Part model, mm, in its own coordinate system. Face numbers are marked on the shaded views. A direction names the side the tool comes from. Give positions to 0.01 mm unless a question says otherwise; leave off trailing zeros. Order: outer loops, then holes, each group sorted by start corner. A loop starts at its lowest first (then second) coordinate and runs counter-clockwise, first axis right, second up.
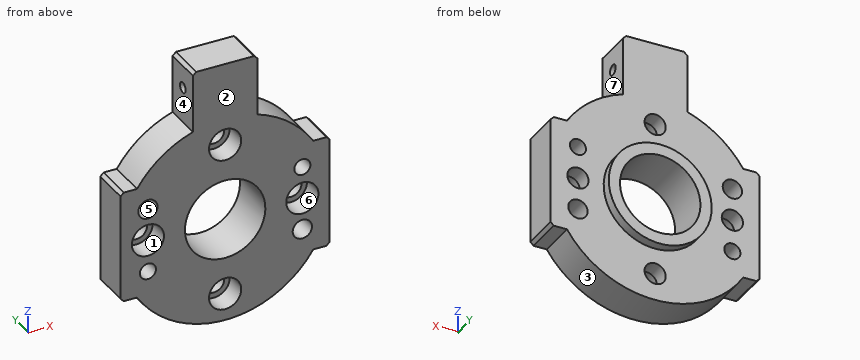
from build123d import *

# Parameters (mm, degrees)
EXTRUDE_1_DEPTH              = 15
SKETCH_2_OUTSIDE_W           = 88.22
SKETCH_2_OUTSIDE_H           = 105.72
SKETCH_2_OUTSIDE_R           = 16
CUT_EXTRUDE_1_DEPTH          = 3
SKETCH_3_R                   = 12.5
CUT_EXTRUDE_2_DEPTH          = 62.491869381
HOLE_WIZARD_M6_1_D           = 6.6
HOLE_WIZARD_M6_1_CBORE_D     = 10
HOLE_WIZARD_M6_1_CBORE_DEPTH = 6.8
F_6_0MM_1_D                  = 6
HOLE_WIZARD_M4_1_D           = 3.3
HOLE_WIZARD_M6_2_D           = 5
CHAMFER_1_SIZE               = 1


with BuildPart() as part:
    # 草图1 → 凸台-拉伸1 (new body)
    with BuildSketch(Plane(origin=(0, 0, 0), x_dir=(1, 0, 0), z_dir=(0, 1, 0))):
        with BuildLine():
            Line((-10, -30.923292192), (-10, -50))
            Line((-10, -50), (10, -50))
            Line((10, -50), (10, -30.923292192))
            ThreePointArc((10, -30.923292192), (19.861440851, -25.724952231), (27.386127875, -17.5))
            Line((27.386127875, -17.5), (32.5, -17.5))
            Line((32.5, -17.5), (32.5, 17.5))
            Line((32.5, 17.5), (27.386127875, 17.5))
            ThreePointArc((27.386127875, 17.5), (0, 32.5), (-27.386127875, 17.5))
            Line((-27.386127875, 17.5), (-32.5, 17.5))
            Line((-32.5, 17.5), (-32.5, -17.5))
            Line((-32.5, -17.5), (-27.386127875, -17.5))
            ThreePointArc((-27.386127875, -17.5), (-19.861440851, -25.724952231), (-10, -30.923292192))
        make_face()
    extrude(amount=EXTRUDE_1_DEPTH)

    # 草图2 outside → 切除-拉伸1 (cut)
    with BuildSketch(Plane(origin=(0, 15, 0), x_dir=(1, 0, 0), z_dir=(0, 1, 0))):
        with Locations((0, -8.75)):
            Rectangle(SKETCH_2_OUTSIDE_W, SKETCH_2_OUTSIDE_H)
        with Locations(Location((0, 0, 0), (0, 0, 270))):
            Circle(SKETCH_2_OUTSIDE_R, mode=Mode.SUBTRACT)
    extrude(amount=-CUT_EXTRUDE_1_DEPTH, mode=Mode.SUBTRACT)

    # 草图3 → 切除-拉伸2 (cut, through all)
    with BuildSketch(Plane.XZ):
        with Locations(Location((0, 0, 0), (0, 0, 270))):
            Circle(SKETCH_3_R)
    extrude(amount=-CUT_EXTRUDE_2_DEPTH, mode=Mode.SUBTRACT)

    # M6 六角圆柱头螺钉的柱形沉头孔1 (through all)
    with Locations(Plane(origin=(0, 0, 0), x_dir=(-1, 0, 0), z_dir=(0, -1, 0))):
        with Locations((0, 24), (24, 0), (0, -24), (-24, 0)):
            CounterBoreHole(HOLE_WIZARD_M6_1_D / 2, HOLE_WIZARD_M6_1_CBORE_D / 2, HOLE_WIZARD_M6_1_CBORE_DEPTH)

    # Ø6.0mm 暗销孔1 (through all)
    with Locations(Plane(origin=(0, 0, 0), x_dir=(-1, 0, 0), z_dir=(0, -1, 0))):
        with Locations((-24, 10), (24, -10)):
            Hole(F_6_0MM_1_D / 2)

    # M4 螺纹孔1 (through all)
    with Locations(Plane.ZY.offset(10)):
        with Locations((42, 6)):
            Hole(HOLE_WIZARD_M4_1_D / 2)

    # M6 螺纹孔2 (through all)
    with Locations(Plane(origin=(0, 0, 0), x_dir=(-1, 0, 0), z_dir=(0, -1, 0))):
        with Locations((24, 10), (-24, -10)):
            Hole(HOLE_WIZARD_M6_2_D / 2)

    # 倒角1
    chamfer_1_edges = [part.edges().sort_by_distance(p)[0] for p in [
        (10, 6, 50),
        (-10, 6, 50),
        (-32.5, 6, 17.5),
        (-32.5, 6, -17.5),
        (32.5, 6, -17.5),
        (32.5, 6, 17.5),
    ]]
    chamfer(chamfer_1_edges, length=CHAMFER_1_SIZE)


solid = part.part
Item 1: Band-saw the part on B-B on z = -10. List the corners of the cut face in (x, y).
Item 2: Band-saw the part on A-A on x = 0. Give the number of separate pieces and of enclosed holes in the cut face, plus the area to 3 significant figures.
Item 3: Drill centre lines: probe 1 along X at (y, z) = (11.75, 1.5); probe 2 along Y at (x, z) = (-0.75, 42); probe 3 along X at (y, z) = (3, -10.5). Where is each one in solid material? Low to high.
Item 4: Band-saw the part on D-D on x = -24. List the corners of the cut face in (y, z), plus the area to 3 significant figures.
Item 5: Pull direction X, two halves, no side cores. Call the marked faces 1, 2 and 3: released by +X, released by -X, zero draft, split by the parting line, or undercut.
Item 6: Drop flat-ended pins along their axis: P1, Ø2, axis at x = -29.5, y = 3.5, coming from the -Z side; P2, Ø8.5, axis at x = 0, z = -24, coming from the +Y side; P3, Ø6, axis at x = 19, y = 5.5, coming from the -Z side; P4, Ø3, axis at x = 12.5, z = 36.5, coming from the -Y side. Give the stop position or say it passes through.
Item 7: Which spindle directions (+Z, -Z, +X, -X, +Y, -Y) get a long thin tool onto all of the face, cutting with end or side? Do the marked faces 4, 5, 6 and 7. Say none if no direction does.
Working result:
1. outline: (-32.5, 0) - (-26.5, 0) - (-26.5, 12) - (-32.5, 12) - close; (-21.5, 0) - (-7.5, 0) - (-7.5, 15) - (-12.49, 15) - (-12.49, 12) - (-21.5, 12) - close; (7.5, 0) - (21, 0) - (21, 12) - (12.49, 12) - (12.49, 15) - (7.5, 15) - close; (27, 0) - (32.5, 0) - (32.5, 12) - (27, 12) - close
2. separate pieces: 4
2. enclosed holes: 1
2. area: 498 mm2
3. probe 1: x = -32.5 to -26.94, -21.06 to -12.41, 12.41 to 21.06, 26.94 to 32.5
3. probe 2: y = 0 to 4.35, 7.65 to 12
3. probe 3: x = -32.5 to -26.45, -21.55 to -6.78, 6.78 to 21.04, 26.96 to 32.5
4. outline: (0, -21.91) - (12, -21.91) - (12, -12.5) - (0, -12.5) - close; (0, -7.5) - (12, -7.5) - (12, -3.3) - (6.8, -3.3) - (6.8, -5) - (0, -5) - close; (0, 5) - (6.8, 5) - (6.8, 3.3) - (12, 3.3) - (12, 7) - (0, 7) - close; (0, 13) - (12, 13) - (12, 21.91) - (0, 21.91) - close
4. area: 292 mm2
5. face 1: undercut
5. face 2: zero draft
5. face 3: split by the parting line
6. P1: stops at z = -17.5
6. P2: stops at y = 12
6. P3: stops at z = -28.29
6. P4: passes through
7. face 4: +Z, -X, +Y, -Y
7. face 5: +Y, -Y
7. face 6: -Y
7. face 7: +Z, +X, +Y, -Y
